Verification items for the finished model (mm, model axes). Give positions to 0.01 mm unless a question says otherwise; leave off trailing zeros. Order: outer loops, then holes, each group sorted by start corner. A loop starts at its lowest first (then second) coordinate and runs counter-clockwise, first axis right, second up.
from build123d import *

# Parameters (mm, degrees)
SKETCH_1_W          = 49
SKETCH_1_H          = 49
EXTRUDE_1_DEPTH     = 10
SKETCH_2_R          = 2.75
CUT_EXTRUDE_1_DEPTH = 71.014284257
HOLE_WIZARD_M12_1_D = 10.2


with BuildPart() as part:
    # 草图1 → 拉伸1 (new body)
    with BuildSketch(Plane(origin=(0, 0, 0), x_dir=(1, 0, 0), z_dir=(0, 1, 0))):
        with Locations((24.5, 24.5)):
            Rectangle(SKETCH_1_W, SKETCH_1_H)
    extrude(amount=EXTRUDE_1_DEPTH)

    # 草图2 → 切除-拉伸1 (cut, through all)
    with BuildSketch(Plane(origin=(0, 10, 0), x_dir=(-1, 0, 0), z_dir=(0, 1, 0))):
        with Locations(Location((-24.5, -5, 0), (0, 0, 90))):
            Circle(SKETCH_2_R)
        with Locations(Location((-44, -24.5, 0), (0, 0, 90))):
            Circle(SKETCH_2_R)
        with Locations(Location((-24.5, -44, 0), (0, 0, 90))):
            Circle(SKETCH_2_R)
        with Locations(Location((-5, -24.5, 0), (0, 0, 90))):
            Circle(SKETCH_2_R)
    extrude(amount=-CUT_EXTRUDE_1_DEPTH, mode=Mode.SUBTRACT)

    # M12 螺纹孔1 (through all)
    with Locations(Plane(origin=(24.5, 10, -22), x_dir=(0, 0, 1), z_dir=(0, 1, 0))):
        with Locations((0, 0)):
            Hole(HOLE_WIZARD_M12_1_D / 2)


solid = part.part
(1) Release check for a two-part mould opening along Z. For faces 1 (the cylindrical face through (5.121, 5.07, -27.247)), 2 (the flat face through (24, 5, 0)), 3 (the flat face through (24, 10, -30)) record: pulls with the +Z half, pulls with the -Z half, needs draft (parallel to the pull), parting line crosses it, or undercut.
Solved:
face 1: undercut
face 2: pulls with the +Z half
face 3: needs draft
(2) Section check C-C, the plane y = 7.5. Enter the section's corners in (x, z), then the cut area to 3 significant figures.
Solved:
outline: (0, -49) - (49, -49) - (49, 0) - (0, 0) - close; hole circle Ø5.5 at (5, -24.5); hole circle Ø10.2 at (24.5, -22); hole circle Ø5.5 at (24.5, -44); hole circle Ø5.5 at (24.5, -5); hole circle Ø5.5 at (44, -24.5)
area: 2,220 mm2
(3) Section check A-A, the plane z = -5. Enter the section's corners in (x, y).
Solved:
outline: (0, 0) - (21.75, 0) - (21.75, 10) - (0, 10) - close; (27.25, 0) - (49, 0) - (49, 10) - (27.25, 10) - close
(4) Scan lines: line 1 (X direction, y = 5, z = -5); line 2 (X direction, y = 1, z = -24); line 3 (X direction, y = 2, z = -26.5). Record each from-to range of solid material in increasing order.
Solved:
line 1: x = 0 to 21.75, 27.25 to 49
line 2: x = 0 to 2.3, 7.7 to 19.81, 29.19 to 41.3, 46.7 to 49
line 3: x = 0 to 3.11, 6.89 to 22.1, 26.9 to 42.11, 45.89 to 49
(5) Section check B-B, the plane x = 44. Enter the section's corners in (y, z).
Solved:
outline: (0, -49) - (10, -49) - (10, -27.25) - (0, -27.25) - close; (0, -21.75) - (10, -21.75) - (10, 0) - (0, 0) - close
